Job drawing, mm, ordinate dimensions from the low corner. One solid piece. A direction names the side the tool comes from. Round coordinates to 2 decimals unless told otherwise and drop trailing zeros. Write each loop counter-clockwise with the first axis right and the second up, starting at its lowest first coordinate (ties: lowest second). Pieces come first, ordered by that corner, then holes. Notation, with made-up numbers: M 89.5,-18 L 128.5,-18 A34 cw 128.5,20 Z; hole C -23,42.25 d5. An arc over 180 degrees is marked long. Write each question's results on one line, items separated by ' | '. Start each with the question number.
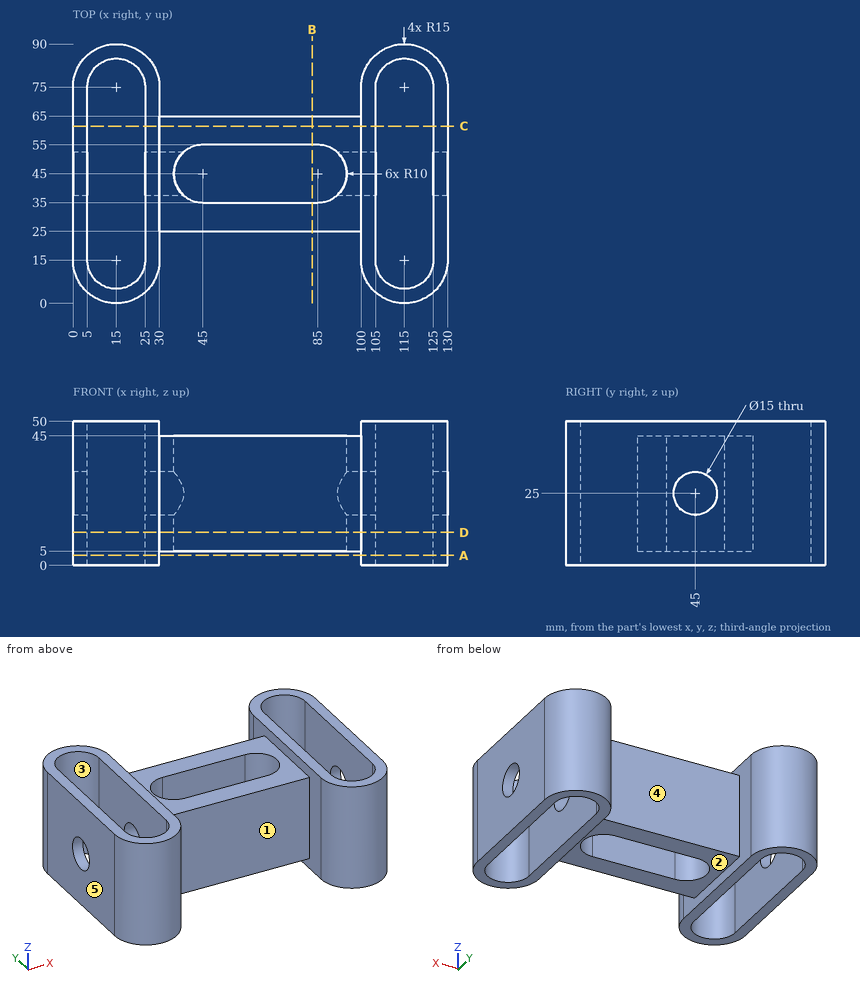
1) Saw through at B-B, the plane x = 83. Write the cut outline in (y, z), plus the area to 3 significant figures.
2) Saw through at A-A, the plane z = 3.5. Write the cut outline in (x, y).
3) Drop flat-ended pins along their axis: pin 1 Ø25 at (y, z) = (49, 19) entering from +X; pin 2 Ø10 at (x, y) = (90, 39.5) entering from -Z; pin 3 Ø20 at (x, z) = (75.5, 17) entering from -Y; pin 4 Ø13.5 at (y, z) = (45, 25) entering from -X. Give the stop position or say it passes through.
4) Saw through at C-C, the plane y = 61.5. Write the cut outline in (x, z), plus the area to 3 significant figures.
5) Saw through at D-D, the plane z = 11.5. Write the cut outline in (x, y), plus the area to 3 significant figures.
6) Wall check: line 1 along X through (y, z) = (55.5, 7); line 2 along X through (y, z) = (73.5, 18); line 3 along Y through (x, z) = (30.5, 25). Give the ranges that are in metal, low to high. Write a range as from..to.
7) Pull direction X, two halves, no side cores. Call the marked faces 4 and 5: pulls with the +X half, pulls with the -X half, needs draft (parallel to the pull), parting line crosses it, or undercut.
8) 3-axis set-ups, long thin cutter, end or side, ignore diameter. For the marked faces 1, 2 and 3: which of +Z, -Z, +X, -X, +Y, -Y reach the whole face in a straight line?
Filled sheet:
1) outline: M 25,5 L 35,5 L 35,45 L 25,45 Z; M 55,5 L 65,5 L 65,45 L 55,45 Z | area: 800 mm^2
2) outline: M 0,15 A15 ccw 30,15 L 30,75 A15 ccw 0,75 Z; M 100,15 A15 ccw 130,15 L 130,75 A15 ccw 100,75 Z; hole M 5,15 A10 ccw 25,15 L 25,75 A10 ccw 5,75 Z; hole M 105,15 A10 ccw 125,15 L 125,75 A10 ccw 105,75 Z
3) pin 1: stops at x = 130 | pin 2: stops at z = 5 | pin 3: stops at y = 25 | pin 4: passes through
4) outline: M 0,0 L 5,0 L 5,50 L 0,50 Z; M 25,0 L 30,0 L 30,5 L 100,5 L 100,0 L 105,0 L 105,50 L 100,50 L 100,45 L 30,45 L 30,50 L 25,50 Z; M 125,0 L 130,0 L 130,50 L 125,50 Z | area: 3,800 mm^2
5) outline: M 0,15 A15 ccw 30,15 L 30,25 L 100,25 L 100,15 A15 ccw 130,15 L 130,75 A15 ccw 100,75 L 100,65 L 30,65 L 30,75 A15 ccw 0,75 Z; hole M 5,15 A10 ccw 25,15 L 25,75 A10 ccw 5,75 Z; hole M 45,35 L 85,35 A10 ccw 85,55 L 45,55 A10 ccw Z; hole M 105,15 A10 ccw 125,15 L 125,75 A10 ccw 105,75 Z | area: 3,670 mm^2
6) line 1: x = 0..5, 25..105, 125..130 | line 2: x = 0..5, 25..30, 100..105, 125..130 | line 3: y = 25..37.5, 52.5..65
7) face 4: undercut | face 5: pulls with the -X half
8) face 1: +Z, -Z, -Y | face 2: -Z, +Y, -Y | face 3: +Z, -Z
